Geometry check sheet. Reference: the model listing, model coordinates, mm. Give positions to 0.01 mm unless a question says otherwise; leave off trailing zeros. Loops run counter-clockwise (first coordinate to the right, second up) from the corner with the lowest first, then second, coordinate; pieces in that order, holes last.
1. Material ranges on L1, parallel to Y at x = 0, z = 1; L2, parallel to Y at x = 21, z = 1.2; L3, parallel to X at y = -17, z = 1.85, recorded low to high.
2. Release check for a two-part mould opening along Y. For faces 1 (the flat face through (0, 0, 0)), 2 (the cylindrical face through (9.793, -4.513, 0.986)) record: +Y half, -Y half, draft (parallel to the pull), parting line (faces both ways), or undercut.
3. Cross-section at B-B, the plane x = 16. Record the cut outline in (y, z).
4. Go/stop test with flat-tipped pins: pin 1 Ø1 at (y, z) = (13.5, 1) entering from +X; pin 2 Ø1 at (x, z) = (-15, 0.5) entering from -Y; pin 3 Ø3.5 at (x, y) = (-21, 0) entering from -Z; pin 4 Ø1 at (y, z) = (14.5, 1) entering from -X. Record where each tip stops, or that it passes through.
5. Cross-section at D-D, the plane z = 0.45. State how many separate pieces and enclosed holes the cut face has, plus the area to 3 significant figures.
6. Cross-section at C-C, the plane y = 10.5. Record the cut outline in (x, z), plus the area to 3 significant figures.
7. Cross-section at A-A, the plane y = 0. Record the cut outline in (x, z).
from build123d import *

# Parameters (mm, degrees)
SKETCH_1_R          = 30
EXTRUDE_1_DEPTH     = 2
SKETCH_2_R          = 1.6
CUT_EXTRUDE_1_DEPTH = 10
SKETCH_3_R          = 2.55
CUT_EXTRUDE_2_DEPTH = 10


with BuildPart() as part:
    # 草图1 → 凸台-拉伸1 (new body)
    with BuildSketch(Plane.XY):
        Circle(SKETCH_1_R)
        with BuildLine():
            Line((4, 16.733200531), (4, 12))
            ThreePointArc((4, 12), (4.527864045, 9.763932023), (6, 8))
            ThreePointArc((6, 8), (7.071067812, 7.071067812), (8, 6))
            ThreePointArc((8, 6), (9.763932023, 4.527864045), (12, 4))
            Line((12, 4), (16.733200531, 4))
            ThreePointArc((16.733200531, 4), (21.025175907, 6.43505412), (21.136674355, 11.368421053))
            ThreePointArc((21.136674355, 11.368421053), (16.970562748, 16.970562748), (11.368421053, 21.136674355))
            ThreePointArc((11.368421053, 21.136674355), (6.43505412, 21.025175907), (4, 16.733200531))
        make_face(mode=Mode.SUBTRACT)
        with BuildLine():
            Line((-4, 16.733200531), (-4, 12))
            ThreePointArc((-4, 12), (-4.527864045, 9.763932023), (-6, 8))
            ThreePointArc((-6, 8), (-7.071067812, 7.071067812), (-8, 6))
            ThreePointArc((-8, 6), (-9.763932023, 4.527864045), (-12, 4))
            Line((-12, 4), (-16.733200531, 4))
            ThreePointArc((-16.733200531, 4), (-21.025175907, 6.43505412), (-21.136674355, 11.368421053))
            ThreePointArc((-21.136674355, 11.368421053), (-16.970562748, 16.970562748), (-11.368421053, 21.136674355))
            ThreePointArc((-11.368421053, 21.136674355), (-6.43505412, 21.025175907), (-4, 16.733200531))
        make_face(mode=Mode.SUBTRACT)
        with BuildLine():
            Line((16.733200531, -4), (12, -4))
            ThreePointArc((12, -4), (9.763932023, -4.527864045), (8, -6))
            ThreePointArc((8, -6), (7.071067812, -7.071067812), (6, -8))
            ThreePointArc((6, -8), (4.527864045, -9.763932023), (4, -12))
            Line((4, -12), (4, -16.733200531))
            ThreePointArc((4, -16.733200531), (6.43505412, -21.025175907), (11.368421053, -21.136674355))
            ThreePointArc((11.368421053, -21.136674355), (16.970562748, -16.970562748), (21.136674355, -11.368421053))
            ThreePointArc((21.136674355, -11.368421053), (21.025175907, -6.43505412), (16.733200531, -4))
        make_face(mode=Mode.SUBTRACT)
        with BuildLine():
            Line((-4, -16.733200531), (-4, -12))
            ThreePointArc((-4, -12), (-4.527864045, -9.763932023), (-6, -8))
            ThreePointArc((-6, -8), (-7.071067812, -7.071067812), (-8, -6))
            ThreePointArc((-8, -6), (-9.763932023, -4.527864045), (-12, -4))
            Line((-12, -4), (-16.733200531, -4))
            ThreePointArc((-16.733200531, -4), (-21.025175907, -6.43505412), (-21.136674355, -11.368421053))
            ThreePointArc((-21.136674355, -11.368421053), (-16.970562748, -16.970562748), (-11.368421053, -21.136674355))
            ThreePointArc((-11.368421053, -21.136674355), (-6.43505412, -21.025175907), (-4, -16.733200531))
        make_face(mode=Mode.SUBTRACT)
    extrude(amount=EXTRUDE_1_DEPTH)

    # 草图2 → 切除-拉伸1 (cut)
    with BuildSketch(Plane.XY.offset(2)):
        with Locations((-21, 0)):
            Circle(SKETCH_2_R)
        with Locations((0, 21)):
            Circle(SKETCH_2_R)
        with Locations((21, 0)):
            Circle(SKETCH_2_R)
        with Locations((0, -21)):
            Circle(SKETCH_2_R)
    extrude(amount=-CUT_EXTRUDE_1_DEPTH, mode=Mode.SUBTRACT)

    # 草图3 → 切除-拉伸2 (cut)
    with BuildSketch(Plane.XY.offset(2)):
        with Locations((0, 6)):
            Circle(SKETCH_3_R)
        with Locations((-6, 0)):
            Circle(SKETCH_3_R)
        with Locations((6, 0)):
            Circle(SKETCH_3_R)
        with Locations((0, -6)):
            Circle(SKETCH_3_R)
    extrude(amount=-CUT_EXTRUDE_2_DEPTH, mode=Mode.SUBTRACT)


solid = part.part
Result:
1. L1: y = -30 to -22.6, -19.4 to -8.55, -3.45 to 3.45, 8.55 to 19.4, 22.6 to 30
1. L2: y = -21.42 to -11.62, -6.39 to -1.6, 1.6 to 6.39, 11.62 to 21.42
1. L3: x = -24.72 to -16.94, -4.01 to 4.01, 16.94 to 24.72
2. face 1: draft
2. face 2: undercut
3. outline: (-25.38, 0) - (-17.89, 0) - (-17.89, 2) - (-25.38, 2) - close; (-4, 0) - (4, 0) - (4, 2) - (-4, 2) - close; (17.89, 0) - (25.38, 0) - (25.38, 2) - (17.89, 2) - close
4. pin 1: stops at x = 27.04
4. pin 2: stops at y = -26.26
4. pin 3: stops at z = 0
4. pin 4: stops at x = -26.53
5. separate pieces: 1
5. enclosed holes: 12
5. area: 1,780 mm2
6. outline: (-28.1, 0) - (-21.5, 0) - (-21.5, 2) - (-28.1, 2) - close; (-4.23, 0) - (4.23, 0) - (4.23, 2) - (-4.23, 2) - close; (21.5, 0) - (28.1, 0) - (28.1, 2) - (21.5, 2) - close
6. area: 43.3 mm2
7. outline: (-30, 0) - (-22.6, 0) - (-22.6, 2) - (-30, 2) - close; (-19.4, 0) - (-8.55, 0) - (-8.55, 2) - (-19.4, 2) - close; (-3.45, 0) - (3.45, 0) - (3.45, 2) - (-3.45, 2) - close; (8.55, 0) - (19.4, 0) - (19.4, 2) - (8.55, 2) - close; (22.6, 0) - (30, 0) - (30, 2) - (22.6, 2) - close
